The listing builds one solid part. Answer for the finished solid, in the listing's coordinates (mm). A direction names the side the tool comes from. Coordinates: 2 decimals unless noted, no trailing zeros. Order: outer loops, then holes, each group sorted by start corner. A loop starts at its lowest first (then second) coordinate and runs counter-clockwise, first axis right, second up. Notation, with made-up numbers: (5, 63.5) -> (35, 63.5) arc R31 cw to (35, 92.5) -> close; hole circle Ø11 at (31, -25.5). An arc over 180 degrees is marked (long way). Write item = value, one per line.
from build123d import *

# Parameters (mm, degrees)
BASE_BLOCK_DEPTH        = 45
STEP_BOSS_PROFILE_W     = 15
STEP_BOSS_PROFILE_H     = 35
STEP_BOSS_DEPTH         = 15
ARM_PROFILE_W           = 30
ARM_PROFILE_H           = 15
EXTENSION_ARM_DEPTH     = 95
HINGE_LUG_PROFILE_R     = 7.5
HINGE_LUG_DEPTH         = 30
EDGE_FILLET_R10_R       = 10
PIN_HOLES_PROFILE_R     = 5
PIN_HOLES_THROUGH_DEPTH = 60
TOP_HOLES_PROFILE_R     = 3.862710878
TOP_HOLES_PROFILE_R_2   = 4.740282405
TOP_HOLES_THROUGH_DEPTH = 60


with BuildPart() as part:
    # Base Block Profile → Base Block (new, symmetric)
    with BuildSketch(Plane.XY):
        Polygon((0, 0), (0, -40), (16, -40), (16, -15), (80, -15), (65, 0), align=None)
    extrude(amount=BASE_BLOCK_DEPTH, both=True)

    # Step Boss Profile → Step Boss (add)
    with BuildSketch(Plane(origin=(0, 0, 0), x_dir=(1, 0, 0), z_dir=(0, 1, 0))):
        with Locations((72.5, -2.5)):
            Rectangle(STEP_BOSS_PROFILE_W, STEP_BOSS_PROFILE_H)
    extrude(amount=-STEP_BOSS_DEPTH)

    # Arm Profile → Extension Arm (add)
    with BuildSketch(Plane(origin=(80, 0, 0), x_dir=(0, 0, -1), z_dir=(1, 0, 0))):
        with Locations((0, -7.5)):
            Rectangle(ARM_PROFILE_W, ARM_PROFILE_H)
    extrude(amount=EXTENSION_ARM_DEPTH)

    # Hinge Lug Profile → Hinge Lug (add)
    with BuildSketch(Plane.XY.offset(15)):
        with BuildLine():
            Line((145, 16), (145, -10.792045984))
            Line((145, -10.792045984), (175, -10.792045984))
            Line((175, -10.792045984), (175, 16))
            ThreePointArc((175, 16), (160, 31), (145, 16))
        make_face()
        with Locations((160, 16)):
            Circle(HINGE_LUG_PROFILE_R, mode=Mode.SUBTRACT)
    extrude(amount=-HINGE_LUG_DEPTH)

    # Edge Fillet R10
    edge_fillet_r10_edges = [part.edges().sort_by_distance(p)[0] for p in [
        (8, -40, 45),
        (8, -40, -45),
    ]]
    fillet(edge_fillet_r10_edges, radius=EDGE_FILLET_R10_R)

    # Pin Holes Profile → Pin Holes Through (cut, symmetric)
    with BuildSketch(Plane.ZY):
        with Locations(Location((-35, -30, 0), (0, 0, 270))):
            Circle(PIN_HOLES_PROFILE_R)
        with Locations(Location((35, -30, 0), (0, 0, 270))):
            Circle(PIN_HOLES_PROFILE_R)
    extrude(amount=PIN_HOLES_THROUGH_DEPTH, both=True, mode=Mode.SUBTRACT)

    # Top Holes Profile → Top Holes Through (cut, symmetric)
    with BuildSketch(Plane(origin=(0, 0, 0), x_dir=(1, 0, 0), z_dir=(0, 1, 0))):
        with Locations(Location((30, 0, 0), (0, 0, 180))):
            Circle(TOP_HOLES_PROFILE_R)
        with Locations(Location((55, 0, 0), (0, 0, 180))):
            Circle(TOP_HOLES_PROFILE_R_2)
    extrude(amount=TOP_HOLES_THROUGH_DEPTH, both=True, mode=Mode.SUBTRACT)


solid = part.part
Q1. Section A-A, the plane x = 30 is taken. Give the vertices of the cut face in (y, z).
The answers:
outline = (-15, -45) -> (0, -45) -> (0, -3.86) -> (-15, -3.86) -> close; (-15, 3.86) -> (0, 3.86) -> (0, 45) -> (-15, 45) -> close
Q2. Find the intervals of material crossed by line 1 along Z through (x, y) = (8, -30); line 2 along Y through (x, z) = (160, 6); line 3 along X through (y, z) = (-18.5, 27), in increasing order.
The answers:
line_1 = -45 to -40, -30 to 30, 40 to 45
line_2 = -15 to 8.5, 23.5 to 31
line_3 = 0 to 16
Q3. The mould has two halves that part along X. Classify faces 1 (the face through (145, 8, 0)), 2 (the face through (59.736, -7.395, 0.208)), 3 (the face through (73, -8, -30)), 4 (the face through (8, -40, 0)): released by +X, released by -X, zero draft, split by the parting line, or undercut.
The answers:
face_1 = released by -X
face_2 = undercut
face_3 = released by +X
face_4 = zero draft
Q4. Section B-B, the plane z = -2 is taken. Give the vertices of the cut face in (x, y), plus the area to 3 significant figures.
The answers:
outline = (0, -40) -> (16, -40) -> (16, -15) -> (26.7, -15) -> (26.7, 0) -> (0, 0) -> close; (33.3, -15) -> (50.7, -15) -> (50.7, 0) -> (33.3, 0) -> close; (59.3, -15) -> (175, -15) -> (175, 16) arc R15 ccw to (145, 16) -> (145, 0) -> (59.3, 0) -> close; hole circle Ø15 at (160, 16)
area = 3,450 mm2
Q5. Each of these flat-tipped pins is pushed along its axis until it touches: pin 1 Ø5 at (y, z) = (-15, 24) entering from +X; pin 2 Ø16 at (y, z) = (-30, -35) entering from +X; pin 3 Ø11 at (x, z) = (55, 0) entering from +Y; pin 4 Ø12 at (x, y) = (75.5, -7.5) entering from +Z. Where does it stop, or does it pass through?
The answers:
pin_1 = 80
pin_2 = 16
pin_3 = 0
pin_4 = 45
Q6. A tool of negligible diameter and unlimited length cuts with its end or side. For faces 5 (the face through (137, -2, 15)), 6 (the face through (8, -25, 35)), 7 (the face through (76, -4, 20)), 8 (the face through (55, 0, -9)), 9 (the face through (77, -15, 1)), from which of +Z, -Z, +X, -X, +Y, -Y can it reach the whole face along a straight path? Write none if from no direction.
The answers:
face_5 = +Z, +X, +Y, -Y
face_6 = +X, -X
face_7 = +Z, +X, +Y
face_8 = +Z, -Z, -X, +Y
face_9 = +Z, -Z, +X, -Y
Q7. Section D-D, the plane x = 11 is taken. Give the vertices of the cut face in (y, z).
The answers:
outline = (-40, -35) arc R10 ccw to (-30, -45) -> (0, -45) -> (0, 45) -> (-30, 45) arc R10 ccw to (-40, 35) -> close; hole circle Ø10 at (-30, -35); hole circle Ø10 at (-30, 35)
Q8. Section C-C, the plane y = -5.5 is taken. Give the vertices of the cut face in (x, z), plus the area to 3 significant figures.
The answers:
outline = (0, -45) -> (70.5, -45) -> (70.5, -15) -> (175, -15) -> (175, 15) -> (80, 15) -> (80, 20) -> (70.5, 20) -> (70.5, 45) -> (0, 45) -> close; hole circle Ø7.73 at (30, 0); hole circle Ø9.48 at (55, 0)
area = 9,410 mm2
